Part model, mm, in its own coordinate system. A direction names the side the tool comes from. Give positions to 0.01 mm unless a question says otherwise; leave off trailing zeros. Order: outer loops, then holes, each group sorted by start corner. A loop starts at its lowest first (then second) coordinate and runs counter-clockwise, first axis right, second up. Notation, with made-up numbers: M -36,-6 L -7,-6 A19 cw -7,24 Z; hole C 80.25,18.5 d8. An arc over 180 degrees is marked long. Answer as a JSON object with one key per item and string values.
from build123d import *

# Parameters (mm, degrees)
SKETCH1_W           = 40
SKETCH1_H           = 180
SKETCH1_R           = 11
BOSS_EXTRUDE1_DEPTH = 16
SKETCH2_R           = 22
BOSS_EXTRUDE2_DEPTH = 20
FILLET1_R           = 5


with BuildPart() as part:
    # Sketch1 → Boss-Extrude1 (new body)
    with BuildSketch(Plane(origin=(0, 0, 0), x_dir=(1, 0, 0), z_dir=(0, 1, 0))):
        Rectangle(SKETCH1_W, SKETCH1_H)
        with Locations(Location((0, 70, 0), (0, 0, 270))):
            Circle(SKETCH1_R, mode=Mode.SUBTRACT)
        with Locations(Location((0, -70, 0), (0, 0, 90))):
            Circle(SKETCH1_R, mode=Mode.SUBTRACT)
    extrude(amount=BOSS_EXTRUDE1_DEPTH)

    # Sketch2 → Boss-Extrude2 (add, symmetric)
    with BuildSketch(Plane(origin=(0, 0, 0), x_dir=(0, 0, -1), z_dir=(1, 0, 0))):
        with BuildLine():
            Line((-42.5, 46), (-42.5, 16))
            Line((-42.5, 16), (42.5, 16))
            Line((42.5, 16), (42.5, 46))
            ThreePointArc((42.5, 46), (0, 88.5), (-42.5, 46))
        make_face()
        with Locations((0, 46)):
            Circle(SKETCH2_R, mode=Mode.SUBTRACT)
    extrude(amount=BOSS_EXTRUDE2_DEPTH, both=True)

    # Fillet1
    fillet1_edges = [part.edges().sort_by_distance(p)[0] for p in [
        (0, 16, 42.5),
        (20, 8, 90),
        (-20, 8, 90),
        (20, 8, -90),
        (-20, 8, -90),
        (0, 16, -42.5),
    ]]
    fillet(fillet1_edges, radius=FILLET1_R)


solid = part.part
1. Which spindle directions (+Z, -Z, +X, -X, +Y, -Y) get a long thin tool onto all of the face, cutting with end or side? Do faces 1 (the flat face through (-5, 16, -60)), 2 (the flat face through (-9.2, 16, 63.7)), 3 (the cylindrical face through (0.28, 88.49, -0.93)). Say none if no direction does.
Worked answers:
{"face 1": "-Z, +X, -X, +Y", "face 2": "+Z, +X, -X, +Y", "face 3": "+X, -X, +Y"}
2. Pin check, flat tips, straight feed: P1, Ø2, axis at x = 16, y = 69.5, coming from the -Z side; P2, Ø10, axis at x = -9, z = 30.5, coming from the +Y side; P3, Ø4, axis at x = -2, z = -17, coming from the +Y side; P4, Ø10, axis at x = 3, z = 50, coming from the -Y side. Stop position of each tip, or through.
Worked answers:
{"P1": "stops at z = -36.06", "P2": "stops at y = 80", "P3": "stops at y = 85.76", "P4": "stops at y = 0"}
3. Cut at C-C on y = 38.5. Give the cut face in (x, z).
Worked answers:
{"outline": "M -20,-42.5 L 20,-42.5 L 20,-20.68 L -20,-20.68 Z; M -20,20.68 L 20,20.68 L 20,42.5 L -20,42.5 Z"}
4. Cut at D-D on x = 17.5. Give the cut face in (y, z).
Worked answers:
{"outline": "M 0,-89.33 L 16,-89.33 L 16,-47.5 A5 cw 21,-42.5 L 46,-42.5 A42.5 ccw 46,42.5 L 21,42.5 A5 cw 16,47.5 L 16,89.33 L 0,89.33 Z; hole C 46,0 d44"}
5. Probe line 1 along X through (y, z) = (3, 70); line 2 along Z through (x, y) = (-7, 14); line 3 along Z through (x, y) = (-14.5, 45). List the from-to ranges inside material, lowest first.
Worked answers:
{"line 1": "x = -20 to -11, 11 to 20", "line 2": "z = -90 to -78.49, -61.51 to 61.51, 78.49 to 90", "line 3": "z = -42.5 to -21.98, 21.98 to 42.5"}
6. Cut at B-B on z = -70. Give the cut face in (x, y).
Worked answers:
{"outline": "M -20,0 L -11,0 L -11,16 L -20,16 Z; M 11,0 L 20,0 L 20,16 L 11,16 Z"}
7. Two-plate mould, pull along X, no slides. Class faces 4 (the cylindrical face through (0, 8, -81)), 5 (the cylindrical face through (18, 8, 89)), 6 (the flat face through (0, 33, -42.5)): +X half, -X half, draft (parallel to the pull), parting line (faces both ways), or undercut.
Worked answers:
{"face 4": "undercut", "face 5": "+X half", "face 6": "draft"}
8. Cut at A-A on x = 0. Give the cut face in (y, z).
Worked answers:
{"outline": "M 0,-90 L 16,-90 L 16,-81 L 0,-81 Z; M 0,-59 L 16,-59 L 16,-47.5 A5 cw 21,-42.5 L 46,-42.5 A42.5 ccw 46,42.5 L 21,42.5 A5 cw 16,47.5 L 16,59 L 0,59 Z; M 0,81 L 16,81 L 16,90 L 0,90 Z; hole C 46,0 d44"}
